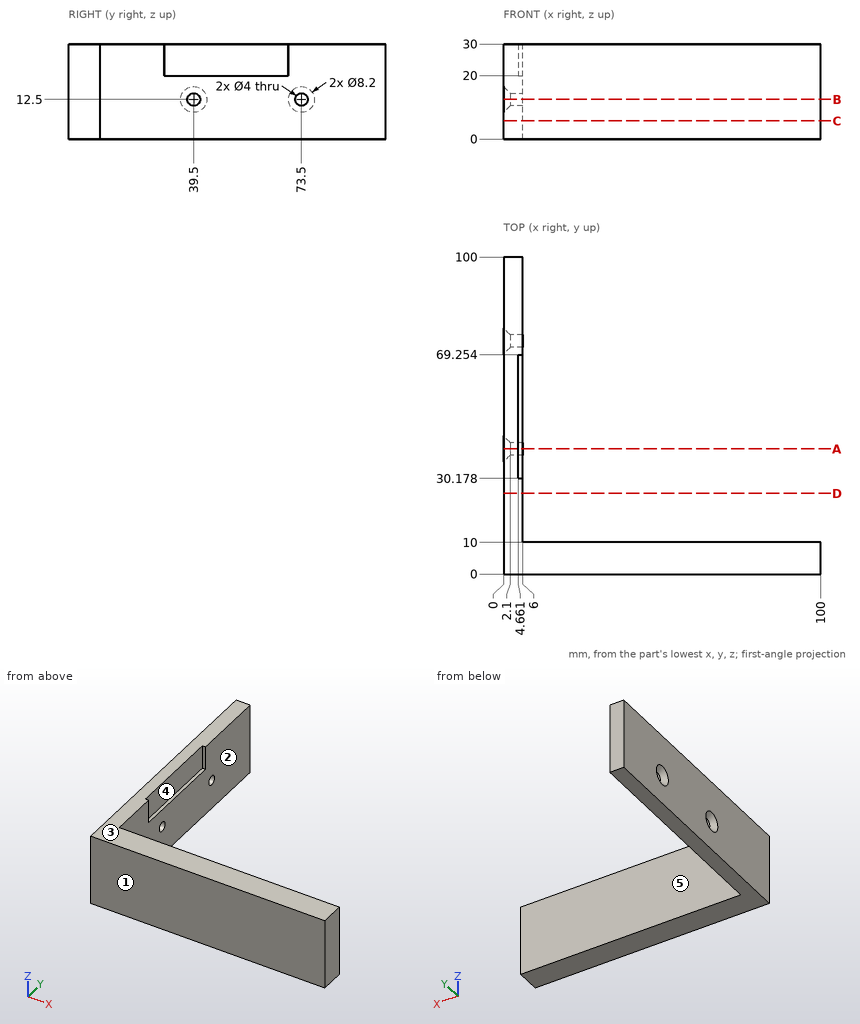
The figure shows three views and two pictorial views of one solid part (mm, origin at its lowest corner). Answer the questions. A direction names the side the tool comes from. Round coordinates to 2 decimals unless told otherwise and drop trailing zeros. Loops run counter-clockwise (first coordinate to the right, second up) from the corner with the lowest first, then second, coordinate; pieces in that order, holes last. Notation, with made-up numbers: M 77,77 L 116,77 A30 ccw 116,106 Z; hole C -18,-29 d6. An arc over 180 degrees is marked long. Write each question's results on one line, items separated by ' | '. Start each with the question number.
1) Find section B-B on z = 12.5. Write down the section's boundary in (x, y), plus the area to 3 significant figures.
2) Find section D-D on y = 25.5. Write down the section's boundary in (x, z).
3) Which of the six approach directions +Z, -Z, +X, -X, +Y, -Y give full straight-line access (tool end or side, diameter ignored) to the marked faces 1 and 2?
4) Straight lines are drawn through the part: probe 1 along Y at (x, z) = (3.8, 12.5); probe 2 along Y at (x, z) = (92, 11.75); probe 3 along X at (y, z) = (29, 10.25). For each, find the intervals that lie inside material, in ascending order.
5) Determine the mould class of the marked faces 3, 4 and 5 for opening direction Y: pulls with the +Y half, pulls with the -Y half, needs draft (parallel to the pull), parting line crosses it, or undercut.
6) Find section A-A on y = 39.5. Write down the section's boundary in (x, z).
7) Each of these flat-tipped pins is pushed along its axis until it touches: pin 1 (15 mm diameter, centred on y = 40, z = 16, fed in from +X); pin 2 (10 mm diameter, centred on x = 78.5, z = 11, fed in from -Y); pin 3 (2 mm diameter, centred on x = 10, z = 11.5, fed in from +Y); pin 4 (2.5 mm diameter, centred on y = 39.5, z = 12.5, fed in from +X). Where does it stop, or does it pass through?
8) Find section C-C on z = 5.75. Write down the section's boundary in (x, y).
Final values:
1) outline: M 0,0 L 100,0 L 100,10 L 6,10 L 6,37.5 L 2.1,37.5 L 0,35.4 Z; M 0,43.6 L 2.1,41.5 L 6,41.5 L 6,71.5 L 2.1,71.5 L 0,69.4 Z; M 0,77.6 L 2.1,75.5 L 6,75.5 L 6,100 L 0,100 Z | area: 1,480 mm²
2) outline: M 0,0 L 6,0 L 6,30 L 0,30 Z
3) face 1: +Z, -Z, +X, -X, -Y | face 2: +Z, -Z, +X, +Y
4) probe 1: 0 to 37.5, 41.5 to 71.5, 75.5 to 100 | probe 2: 0 to 10 | probe 3: 0 to 6
5) face 3: needs draft | face 4: undercut | face 5: pulls with the +Y half
6) outline: M 0,0 L 6,0 L 6,10.5 L 2.1,10.5 L 0,8.4 Z; M 0,16.6 L 2.1,14.5 L 6,14.5 L 6,20 L 4.66,20 L 4.66,30 L 0,30 Z
7) pin 1: x = 6 | pin 2: y = 0 | pin 3: y = 10 | pin 4: through
8) outline: M 0,0 L 100,0 L 100,10 L 6,10 L 6,100 L 0,100 Z
